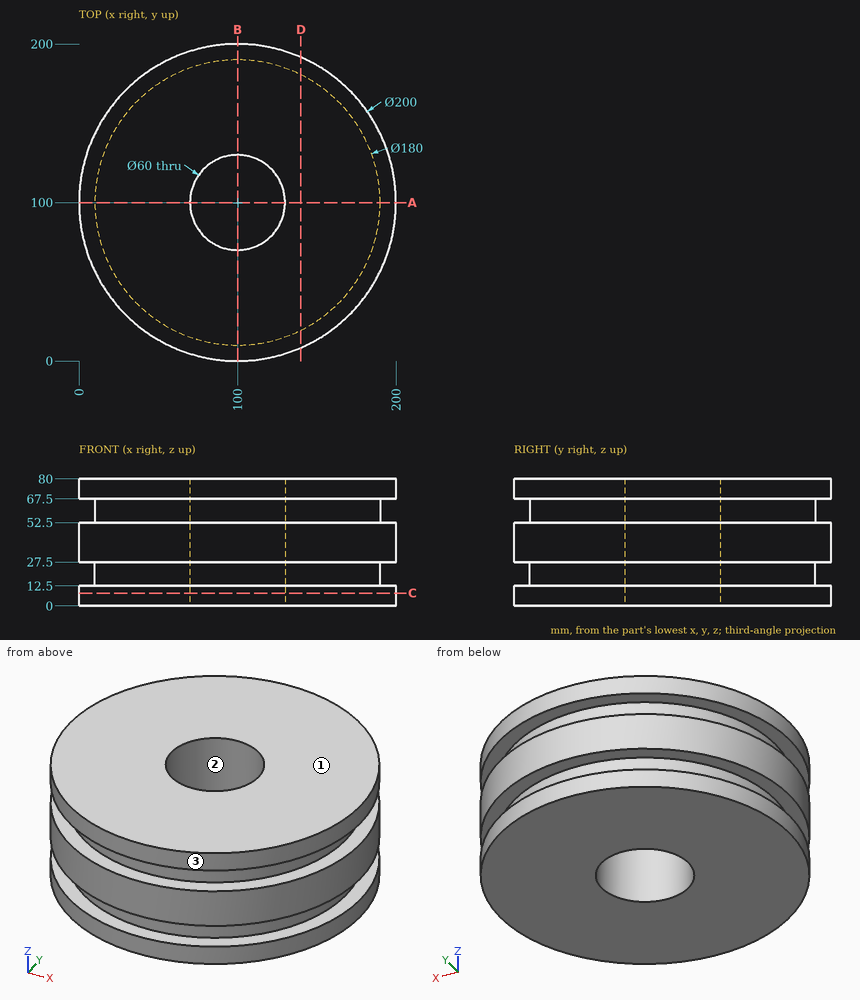
For this review, use the dimensioned drawing (mm, ordinates from the lowest corner) and the shaded views. Give positions to 0.01 mm unless a question says otherwise; leave off trailing zeros. Loops run counter-clockwise (first coordinate to the right, second up) from the corner with the lowest first, then second, coordinate; pieces in that order, holes last. Notation, with made-up numbers: (-25, -20) -> (-13, -20) arc R30 ccw to (-13, 14) -> close; hole circle Ø6 at (57, -6). An arc over 180 degrees is marked (long way). One line per question, with ' | ' between items. Start each with the question number.
(1) We need section C-C (z = 8). State the section outline as (x, y) points.
(2) For line 1 (Z direction, x = 67, y = 11); line 2 (Y direction, x = 100, z = 59); line 3 (Y direction, x = 100, z = 36), list the stretches that pass through material, from the lowest coordinate up.
(3) Insertion check: P1, Ø1, axis at y = 109, z = 71, coming from the -X side; P2, Ø12, axis at x = 112.5, z = 50.5, coming from the -Y side; P3, Ø12, axis at x = 148.5, z = 13, coming from the +Y side. Each pin has a flat end and moves straight along its axis. Give the tip position at first contact, or say it passes through.
(4) We need section D-D (x = 140). State the section outline as (y, z) points.
(5) We need section A-A (y = 100). State the section outline as (x, z) points, and give its area (3 significant figures).
(6) Draft analysis for pull direction Y (two halves, no side actions). For the marked faces 1, 2 and 3, state which applies: +Y half, -Y half, draft (parallel to the pull), parting line (faces both ways), or undercut.
The answers:
1) outline: circle Ø200 at (100, 100); hole circle Ø60 at (100, 100)
2) line 1: z = 0 to 12.5, 27.5 to 52.5, 67.5 to 80 | line 2: y = 10 to 70, 130 to 190 | line 3: y = 0 to 70, 130 to 200
3) P1: stops at x = 0.36 | P2: stops at y = 0.21 | P3: stops at y = 190.51
4) outline: (8.35, 0) -> (191.65, 0) -> (191.65, 12.5) -> (180.62, 12.5) -> (180.62, 27.5) -> (191.65, 27.5) -> (191.65, 52.5) -> (180.62, 52.5) -> (180.62, 67.5) -> (191.65, 67.5) -> (191.65, 80) -> (8.35, 80) -> (8.35, 67.5) -> (19.38, 67.5) -> (19.38, 52.5) -> (8.35, 52.5) -> (8.35, 27.5) -> (19.38, 27.5) -> (19.38, 12.5) -> (8.35, 12.5) -> close
5) outline: (0, 0) -> (70, 0) -> (70, 80) -> (0, 80) -> (0, 67.5) -> (10, 67.5) -> (10, 52.5) -> (0, 52.5) -> (0, 27.5) -> (10, 27.5) -> (10, 12.5) -> (0, 12.5) -> close; (130, 0) -> (200, 0) -> (200, 12.5) -> (190, 12.5) -> (190, 27.5) -> (200, 27.5) -> (200, 52.5) -> (190, 52.5) -> (190, 67.5) -> (200, 67.5) -> (200, 80) -> (130, 80) -> close | area: 10,600 mm^2
6) face 1: draft | face 2: undercut | face 3: parting line
